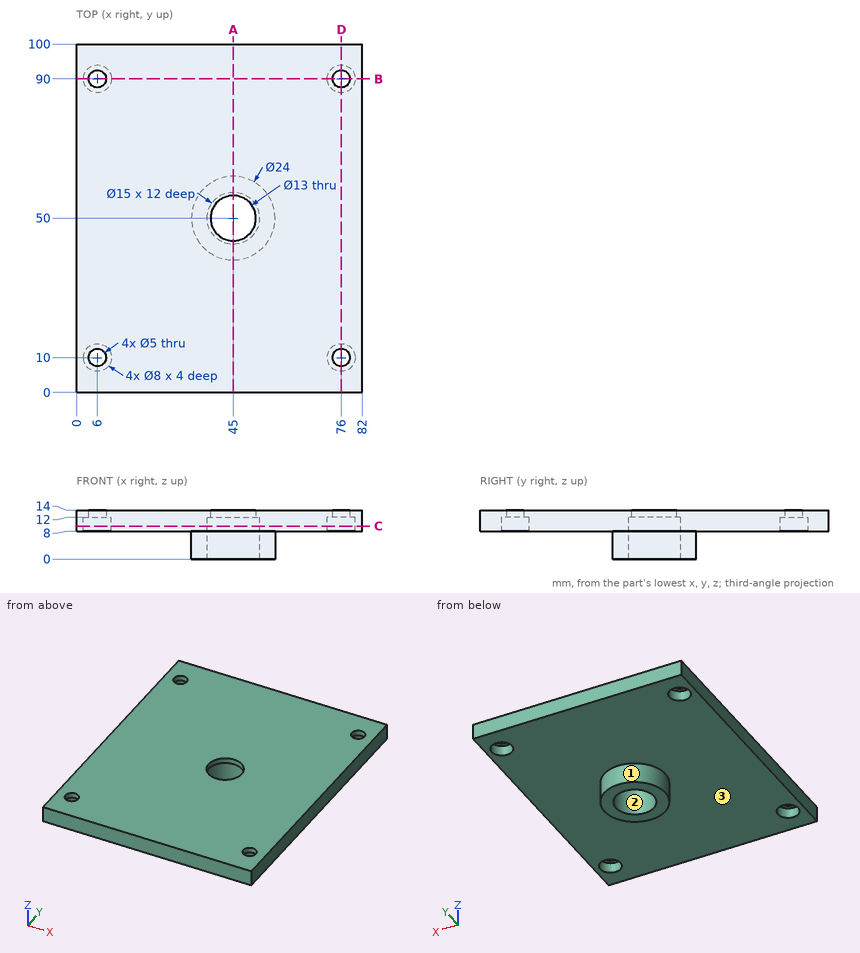
Design review of the part shown in the three views and the two pictorial views. Dimensions are in mm from the part's minimum x, y and z. Round coordinates to 2 decimals unless told otherwise and drop trailing zeros. Write each loop counter-clockwise with the first axis right and the second up, starting at its lowest first coordinate (ties: lowest second). Pieces come first, ordered by that corner, then holes. Notation, with made-up numbers: (34, -30) - (50, -30) arc R34 cw to (50, 4) - close; hole circle Ø4 at (15, 39). An arc over 180 degrees is marked (long way). Write item = value, one per line. Start each with the question number.
1. Consider section D-D on x = 76. State the section outline as (y, z) points.
2. Consider section B-B on y = 90. State the section outline as (x, z) points.
3. For pin 1 Ø4.5 at (x, y) = (6, 90) entering from -Z; pin 2 Ø6.5 at (x, y) = (76, 10) entering from -Z; pin 3 Ø8 at (x, y) = (18, 10) entering from -Z, all flat-tipped, find the tip position at first contact; note any pin that passes through.
4. Consider section A-A on x = 45. State the section outline as (y, z) points.
5. Draft analysis for pull direction X (two halves, no side actions). For the marked faces 1, 2 and 3, state which applies: released by +X, released by -X, zero draft, split by the parting line, or undercut.
6. Wall thickness on L1, parallel to Y at x = 76, z = 11; L2, parallel to Y at x = 6, z = 13.1; L3, parallel to X at y = 90, z = 13.45: over which ranges is each line inside the solid? List them lowest first.
7. Consider section C-C on z = 9.5. State the section outline as (x, y) points, plus the area to 3 significant figures.
Evaluation:
q1.outline = (0, 8) - (6, 8) - (6, 12) - (7.5, 12) - (7.5, 14) - (0, 14) - close; (12.5, 12) - (14, 12) - (14, 8) - (86, 8) - (86, 12) - (87.5, 12) - (87.5, 14) - (12.5, 14) - close; (92.5, 12) - (94, 12) - (94, 8) - (100, 8) - (100, 14) - (92.5, 14) - close
q2.outline = (0, 8) - (2, 8) - (2, 12) - (3.5, 12) - (3.5, 14) - (0, 14) - close; (8.5, 12) - (10, 12) - (10, 8) - (72, 8) - (72, 12) - (73.5, 12) - (73.5, 14) - (8.5, 14) - close; (78.5, 12) - (80, 12) - (80, 8) - (82, 8) - (82, 14) - (78.5, 14) - close
q3.pin_1 = through
q3.pin_2 = 12
q3.pin_3 = 8
q4.outline = (0, 8) - (38, 8) - (38, 0) - (42.5, 0) - (42.5, 12) - (43.5, 12) - (43.5, 14) - (0, 14) - close; (56.5, 12) - (57.5, 12) - (57.5, 0) - (62, 0) - (62, 8) - (100, 8) - (100, 14) - (56.5, 14) - close
q5.face_1 = split by the parting line
q5.face_2 = undercut
q5.face_3 = zero draft
q6.L1 = 0 to 6, 14 to 86, 94 to 100
q6.L2 = 0 to 7.5, 12.5 to 87.5, 92.5 to 100
q6.L3 = 0 to 3.5, 8.5 to 73.5, 78.5 to 82
q7.outline = (0, 0) - (82, 0) - (82, 100) - (0, 100) - close; hole circle Ø8 at (6, 10); hole circle Ø8 at (6, 90); hole circle Ø15 at (45, 50); hole circle Ø8 at (76, 10); hole circle Ø8 at (76, 90)
q7.area = 7,820 mm2
